Here's how the part is built. I have some questions about the finished solid (model axes, mm). A direction names the side the tool comes from. Coordinates: 2 decimals unless noted, no trailing zeros. Write each loop counter-clockwise with the first axis right and the second up, starting at its lowest first coordinate (ties: lowest second). Pieces come first, ordered by that corner, then holes. Notation, with made-up numbers: M 39,69 L 82,69 A34 cw 82,102 Z; hole C -23.75,79.5 d1. An arc over 180 degrees is marked long. Use a Markdown table: item, result.
```python
from build123d import *

# Parameters (mm, degrees)
SKETCH1_R           = 12
BOSS_EXTRUDE1_DEPTH = 22
SKETCH2_R           = 14
BOSS_EXTRUDE2_DEPTH = 96
CUT_EXTRUDE1_START  = -66
SKETCH3_R           = 14
SKETCH3_R_2         = 12.5
CUT_EXTRUDE1_DEPTH  = 66
CHAMFER1_SIZE       = 3
MOVE_FACE1_BY       = 49
CUT_EXTRUDE2_DEPTH  = 3


with BuildPart() as part:
    # Sketch1 → Boss-Extrude1 (new body)
    with BuildSketch(Plane.XY):
        Circle(SKETCH1_R)
    extrude(amount=-BOSS_EXTRUDE1_DEPTH)

    # Sketch2 → Boss-Extrude2 (add)
    with BuildSketch(Plane.XY):
        Circle(SKETCH2_R)
    extrude(amount=BOSS_EXTRUDE2_DEPTH)

    # Sketch3 → Cut-Extrude1 (cut)
    with BuildSketch(Plane.XY.offset(96).offset(CUT_EXTRUDE1_START)):
        Circle(SKETCH3_R)
        Circle(SKETCH3_R_2, mode=Mode.SUBTRACT)
    extrude(amount=CUT_EXTRUDE1_DEPTH, mode=Mode.SUBTRACT)

    # Chamfer1
    chamfer1_edges = [part.edges().sort_by_distance(p)[0] for p in [
        (-12.5, 0, 96),
        (-12, 0, -22),
    ]]
    chamfer(chamfer1_edges, length=CHAMFER1_SIZE)

    # Move Face1: a face moved outward by 49.0
    extrude(part.faces().sort_by_distance((-7, -11.2, 30))[0], amount=MOVE_FACE1_BY, dir=(0, 0, 1))

    # Sketch4 → Cut-Extrude2 (cut)
    with BuildSketch(Plane(origin=(0, 12.5, 0), x_dir=(1, 0, 0), z_dir=(0, 1, 0))):
        with BuildLine():
            Line((-2.5, -90.2), (-2.5, -82.2))
            ThreePointArc((-2.5, -82.2), (0, -79.7), (2.5, -82.2))
            Line((2.5, -82.2), (2.5, -90.2))
            ThreePointArc((2.5, -90.2), (0, -92.7), (-2.5, -90.2))
        make_face()
    extrude(amount=-CUT_EXTRUDE2_DEPTH, mode=Mode.SUBTRACT)


solid = part.part
```
1. Suppose I cut it at A-A on x = 0. Write out the boundary of the cut face in (y, z), and give its area (3 significant figures).
Answers follow:
| item | result |
|---|---|
| outline | M -14,0 L -12,0 L -12,-19 L -9,-22 L 9,-22 L 12,-19 L 12,0 L 14,0 L 14,79 L 12.5,79 L 12.5,79.7 L 9.5,79.7 L 9.5,92.7 L 12.5,92.7 L 12.5,93 L 9.5,96 L -9.5,96 L -12.5,93 L -12.5,79 L -14,79 Z |
| area | 3,110 mm2 |
2. Suppose I cut it at B-B on y = 0. Write out the boundary of the cut face in (x, z), and give its area (3 significant figures).
Answers follow:
| item | result |
|---|---|
| outline | M -14,0 L -12,0 L -12,-19 L -9,-22 L 9,-22 L 12,-19 L 12,0 L 14,0 L 14,79 L 12.5,79 L 12.5,93 L 9.5,96 L -9.5,96 L -12.5,93 L -12.5,79 L -14,79 Z |
| area | 3,150 mm2 |
3. Suppose I cut it at D-D on z = -9. Write out the boundary of the cut face in (x, y).
Answers follow:
| item | result |
|---|---|
| outline | C 0,0 d24 |
4. I need wall thicknesses on probe 1 along X at (y, z) = (6.25, 73); probe 2 along Y at (x, z) = (0.5, 30); probe 3 along Z at (x, y) = (11.5, -5). Which ranges of each line are inside material? Lowest first, please.
Answers follow:
| item | result |
|---|---|
| probe 1 | x = -12.53 to 12.53 |
| probe 2 | y = -13.99 to 13.99 |
| probe 3 | z = 0 to 79 |
5. Will these pins go through, and if not, where does the flat tip stop? pin 1 Ø3 at (y, z) = (8.5, 70.5) entering from -X; pin 2 Ø10 at (x, z) = (-10.5, 34) entering from -Y; pin 3 Ø8 at (x, z) = (5, -5) entering from -Y.
Answers follow:
| item | result |
|---|---|
| pin 1 | stops at x = -12.12 |
| pin 2 | stops at y = -12.87 |
| pin 3 | stops at y = -11.96 |
6. Which directions (+Z, -Z, +X, -X, +Y, -Y) give clear straight access to the entire face, cutting with the end or side of a thin tool? Please do faces 4 (the face through (5.77, -11.09, 85.9)), 5 (the face through (0, 0, -22)), 6 (the face through (-11.99, 0.53, -9.37)), 7 (the face through (0.1, 11, 92.7)).
Answers follow:
| item | result |
|---|---|
| face 4 | +Z |
| face 5 | -Z, +X, -X, +Y, -Y |
| face 6 | -Z |
| face 7 | +Y |
7. We'd pull the mould along Z, two halves only. Please class faces 1 (the face through (12.932, -5.362, 38.947)), 2 (the face through (-0.1, 11, 79.7)), 3 (the face through (-6.3, 10.4, 0)): +Z half, -Z half, draft (parallel to the pull), parting line (faces both ways), or undercut.
Answers follow:
| item | result |
|---|---|
| face 1 | draft |
| face 2 | undercut |
| face 3 | -Z half |
8. Suppose I cut it at C-C on z = 55.5. Write out the boundary of the cut face in (x, y).
Answers follow:
| item | result |
|---|---|
| outline | C 0,0 d28 |
